Geometry: final body of the model. Coordinates: model frame, mm. A direction names the side the tool comes from. Round coordinates to 2 decimals unless told otherwise and drop trailing zeros. Loops run counter-clockwise (first coordinate to the right, second up) from the corner with the lowest first, then second, coordinate; pieces in that order, holes last. Notation, with made-up numbers: M 86,69.25 L 91,69.25 A31 cw 91,104.25 Z; hole C 55,-3 d1. An arc over 180 degrees is marked long. Answer as a JSON object with one key per item and string values.
```python
from build123d import *

# Parameters (mm, degrees)
SKETCH1_W           = 70
SKETCH1_H           = 70
BOSS_EXTRUDE1_DEPTH = 70
SKETCH2_W           = 60
SKETCH2_H           = 60
CUT_EXTRUDE1_DEPTH  = 104
SKETCH3_W           = 12.4
SKETCH3_H           = 5.4
CUT_EXTRUDE2_DEPTH  = 10
SKETCH4_R           = 4
CUT_EXTRUDE3_DEPTH  = 122
FILLET1_R           = 5


with BuildPart() as part:
    # Sketch1 → Boss-Extrude1 (new body)
    with BuildSketch(Plane.XY):
        Rectangle(SKETCH1_W, SKETCH1_H)
    extrude(amount=BOSS_EXTRUDE1_DEPTH)

    # Sketch2 → Cut-Extrude1 (cut)
    with BuildSketch(Plane(origin=(35, 0, 0), x_dir=(0, 0, -1), z_dir=(1, 0, 0))):
        with Locations((-35, 0)):
            Rectangle(SKETCH2_W, SKETCH2_H)
    extrude(amount=-CUT_EXTRUDE1_DEPTH, mode=Mode.SUBTRACT)

    # Sketch3 → Cut-Extrude2 (cut)
    with BuildSketch(Plane(origin=(0, 0, 0), x_dir=(-1, 0, 0), z_dir=(0, 0, -1))):
        Rectangle(SKETCH3_W, SKETCH3_H)
    extrude(amount=-CUT_EXTRUDE2_DEPTH, mode=Mode.SUBTRACT)

    # Sketch4 → Cut-Extrude3 (cut)
    with BuildSketch(Plane.XZ.offset(35)):
        with Locations(Location((0, 35, 0), (0, 0, 270))):
            Circle(SKETCH4_R)
    extrude(amount=-CUT_EXTRUDE3_DEPTH, mode=Mode.SUBTRACT)

    # Fillet1
    fillet1_edges = [part.edges().sort_by_distance(p)[0] for p in [
        (0, 35, 70),
        (0, -30, 5),
        (0, -30, 65),
        (0, 30, 65),
        (0, 30, 5),
        (0, 35, 0),
        (0, -35, 0),
        (0, -35, 70),
    ]]
    fillet(fillet1_edges, radius=FILLET1_R)


solid = part.part
```
1) Pull-direction query (Z, two-part tool) for faces 4 (the face through (0, -6, 5)), 5 (the face through (0, -30, 41)), 6 (the face through (0, -34, 2)), 7 (the face through (35, 0, 66)); classes: +Z half, -Z half, draft (parallel to the pull), parting line (faces both ways), or undercut.
Geometry results:
{"face 4": "undercut", "face 5": "undercut", "face 6": "-Z half", "face 7": "draft"}
2) Line query: probe 1 along Y at (x, z) = (32, 30); probe 2 along Z at (x, y) = (-31, 3); probe 3 along X at (y, z) = (-32, 35). Output: solid intervals per line, ascending.
Geometry results:
{"probe 1": "-35 to -30, 30 to 35", "probe 2": "0 to 5, 65 to 70", "probe 3": "-35 to -4, 4 to 35"}
3) Cut plane B-B on z = 23.5. Return the cut outline in (x, y).
Geometry results:
{"outline": "M -35,-35 L 35,-35 L 35,-30 L -35,-30 Z; M -35,30 L 35,30 L 35,35 L -35,35 Z"}
4) First-contact query: pin 1 (6.5 mm diameter, centred on x = 0, z = 35, fed in from -Y); pin 2 (5.5 mm diameter, centred on x = -1.5, z = 2, fed in from +Y); pin 3 (2.5 mm diameter, centred on x = -2, z = 3, fed in from -Y). Flat tips, straight axial feed; report the tip coordinate or a pass-through.
Geometry results:
{"pin 1": "through", "pin 2": "y = 34.99", "pin 3": "y = -34.94"}
5) Set-up query: faces 1 (the face through (0, -2.7, 2)), 2 (the face through (0, 7, 0)), 3 (the face through (0, 0, 65)). Return all of +Z, -Z, +X, -X, +Y, -Y with unobstructed straight access to the full face (end or side cutting, diameter ignored); none if empty.
Geometry results:
{"face 1": "-Z", "face 2": "-Z, +X, -X, +Y, -Y", "face 3": "+X, -X"}
6) Cut plane C-C on x = 0. Return the cut outline in (y, z).
Geometry results:
{"outline": "M -35,5 A5 ccw -30,0 L -2.7,0 L -2.7,5 L -25,5 A5 cw -30,10 L -30,31 L -35,31 Z; M -35,39 L -30,39 L -30,60 A5 cw -25,65 L 25,65 A5 cw 30,60 L 30,39 L 35,39 L 35,65 A5 ccw 30,70 L -30,70 A5 ccw -35,65 Z; M 2.7,0 L 30,0 A5 ccw 35,5 L 35,31 L 30,31 L 30,10 A5 cw 25,5 L 2.7,5 Z"}
7) Cut plane D-D on z = 35. Return the cut outline in (x, y), and give its area (3 significant figures).
Geometry results:
{"outline": "M -35,-35 L -4,-35 L -4,-30 L -35,-30 Z; M -35,30 L -4,30 L -4,35 L -35,35 Z; M 4,-35 L 35,-35 L 35,-30 L 4,-30 Z; M 4,30 L 35,30 L 35,35 L 4,35 Z", "area": "620 mm2"}
8) Cut plane A-A on y = 15. Return the cut outline in (x, z).
Geometry results:
{"outline": "M -35,0 L 35,0 L 35,5 L -35,5 Z; M -35,65 L 35,65 L 35,70 L -35,70 Z"}
